The listing builds one solid part. Answer for the finished solid, in the listing's coordinates (mm). A direction names the side the tool comes from. Coordinates: 2 decimals unless noted, no trailing zeros. Order: outer loops, then holes, each group sorted by start corner. A loop starts at its lowest first (then second) coordinate and runs counter-clockwise, first axis right, second up. Notation, with made-up numbers: (76.5, 13.5) -> (110.5, 13.5) arc R9 cw to (110.5, 19.5) -> close; hole circle Ø10 at (4.5, -39). An arc over 180 degrees is marked (long way). Write item = value, one per line.
from build123d import *

# Parameters (mm, degrees)
SKETCH2_R           = 15
SKETCH2_R_2         = 9.9
BOSS_EXTRUDE1_DEPTH = 5
SKETCH3_R           = 12
SKETCH3_R_2         = 9.9
BOSS_EXTRUDE2_DEPTH = 10
CHAMFER1_SIZE       = 1


with BuildPart() as part:
    # Sketch2 → Boss-Extrude1 (new body)
    with BuildSketch(Plane.XY):
        Circle(SKETCH2_R)
        Circle(SKETCH2_R_2, mode=Mode.SUBTRACT)
    extrude(amount=BOSS_EXTRUDE1_DEPTH)

    # Sketch3 → Boss-Extrude2 (add)
    with BuildSketch(Plane.XY.offset(5)):
        Circle(SKETCH3_R)
        Circle(SKETCH3_R_2, mode=Mode.SUBTRACT)
    extrude(amount=BOSS_EXTRUDE2_DEPTH)

    # Chamfer1
    chamfer1_edges = [part.edges().sort_by_distance(p)[0] for p in [
        (-12, 0, 15),
        (-15, 0, 0),
        (-15, 0, 5),
    ]]
    chamfer(chamfer1_edges, length=CHAMFER1_SIZE)


solid = part.part
Q1. Section D-D, the plane z = 13.5 is taken. Give the vertices of the cut face in (x, y), plus the area to 3 significant figures.
The answers:
outline = circle Ø24 at (0, 0); hole circle Ø19.8 at (0, 0)
area = 144 mm2
Q2. Each of these flat-tipped pins is pushed along its axis until it touches: pin 1 Ø5 at (x, z) = (2.5, 8.5) entering from +Y; pin 2 Ø8 at (y, z) = (9, 13.5) entering from -X; pin 3 Ø4 at (y, z) = (-7.5, 4) entering from +X. Where does it stop, or does it pass through?
The answers:
pin_1 = 12
pin_2 = -10.91
pin_3 = 13.96
Q3. Find the intervals of material crossed by line 1 along Y through (x, z) = (0, 9.75); line 2 along Z through (x, y) = (13.75, 0.5); line 3 along Y through (x, z) = (-2.75, 10.5), in increasing order.
The answers:
line_1 = -12 to -9.9, 9.9 to 12
line_2 = 0 to 5
line_3 = -11.68 to -9.51, 9.51 to 11.68
Q4. Section A-A, the plane x = 0 is taken. Give the vertices of the cut face in (y, z), plus the area to 3 significant figures.
The answers:
outline = (-15, 1) -> (-14, 0) -> (-9.9, 0) -> (-9.9, 15) -> (-11, 15) -> (-12, 14) -> (-12, 5) -> (-14, 5) -> (-15, 4) -> close; (9.9, 0) -> (14, 0) -> (15, 1) -> (15, 4) -> (14, 5) -> (12, 5) -> (12, 14) -> (11, 15) -> (9.9, 15) -> close
area = 90.0 mm2
Q5. The mould has two halves that part along Y. Classify faces 1 (the face through (-14.985, 0.66, 2.479)), 2 (the face through (3, 10, 0)), 3 (the face through (9.443, 2.974, 7.395)): released by +Y, released by -Y, zero draft, split by the parting line, or undercut.
The answers:
face_1 = split by the parting line
face_2 = zero draft
face_3 = undercut
Q6. A tool of negligible diameter and unlimited length cuts with its end or side. For faces 4 (the face through (-11.99, 0.53, 9.44)), 5 (the face through (-10, 2, 15)), from which of +Z, -Z, +X, -X, +Y, -Y can it reach the whole face along a straight path? Write none if from no direction.
The answers:
face_4 = +Z
face_5 = +Z, +X, -X, +Y, -Y
Q7. Section C-C, the plane z = 2.75 is taken. Give the vertices of the cut face in (x, y).
The answers:
outline = circle Ø30 at (0, 0); hole circle Ø19.8 at (0, 0)
